The model under review builds one solid part; all positions refer to its coordinate system, in mm. A direction names the side the tool comes from. Give positions to 0.01 mm unless a question says otherwise; leave off trailing zeros. Loops run counter-clockwise (first coordinate to the right, second up) from the corner with the lowest first, then second, coordinate; pieces in that order, holes last. Notation, with made-up numbers: (-30, -17.75) -> (5, -17.75) arc R24 cw to (5, -2.75) -> close; hole circle Ø6 at (13, 6). An arc over 180 degrees is marked (long way). Write each question's results on one line, items separated by ' | '. Start each with the question number.
Q1. We need section C-C (y = 65.5). Write out the cut boundary in (x, z), plus the area to 3 significant figures.
Q2. Mouldability with a two-part tool opening along Z and no side actions: class faces 4 (the face through (2, 0, 67)), 5 (the face through (-59.37, 17.26, 143.18)), 6 (the face through (-105.034, 7.605, -66.17)) as released by +Z, released by -Z, zero draft, split by the parting line, or undercut.
Q3. We need section B-B (z = -112.5). Write out the cut boundary in (x, y).
Q4. Wall thickness on L1, parallel to X at y = 23, z = -1; L2, parallel to X at y = 77, z = 0; L3, parallel to X at y = 11.5, z = 0: over which ranges is each line inside the solid? List them lowest first. Write a range as [from, to].
Q5. We need section D-D (z = -56.25). Write out the cut boundary in (x, y), plus the area to 3 significant figures.
Q6. Insertion check: pin 1 Ø2 at (x, z) = (-23.5, 120) entering from +Y; pin 2 Ø3 at (y, z) = (60.5, -43) entering from -X; pin 3 Ø8 at (x, y) = (-1.5, 49.5) entering from +Z. Each pin has a flat end and moves straight along its axis. Give the tip position at first contact, or say it passes through.
Q7. We need section A-A (x = 0). Give the number of separate pieces and of enclosed holes in the cut face, plus the area to 3 significant figures.
Q8. Machinability: for faces 1 (the face through (37, 98, 10)), 2 (the face through (2.64, 24.65, 59.94)), 3 (the face through (-65, 15, 65)), which of the approach directions +Z, -Z, +X, -X, +Y, -Y give a long, thin tool a straight path to every point of the face, cutting with its end or side? Answer none if there is none.
from build123d import *

# Parameters (mm, degrees)
FLANGE_RIM_SKETCH_R              = 155
FLANGE_RIM_SKETCH_R_2            = 150
FLANGE_RIM_310_DEPTH             = 35
FLANGE_BASE_SKETCH_R             = 150
FLANGE_BASE_DISC_DEPTH           = 15
MOUNTING_HOLES_SKETCH_R          = 12.5
MOUNTING_HOLES_6X_DEPTH          = 65
HUB_SHOULDER_SKETCH_R            = 80
HUB_SHOULDER_160_DEPTH           = 25
HUB_SKETCH_R                     = 75
HUB_150_DEPTH                    = 105
KEYED_BORE_WITH_KEYWAY_8X8_DEPTH = 142
RECESS_SKETCH_R                  = 60
RECESS_120_DEPTH                 = 50


with BuildPart() as part:
    # Flange Rim Sketch → Flange Rim Ø310 (new body)
    with BuildSketch(Plane(origin=(0, 0, 0), x_dir=(1, 0, 0), z_dir=(0, 1, 0))):
        with Locations(Location((0, 0, 0), (0, 0, 270))):
            Circle(FLANGE_RIM_SKETCH_R)
        with Locations(Location((0, 0, 0), (0, 0, 270))):
            Circle(FLANGE_RIM_SKETCH_R_2, mode=Mode.SUBTRACT)
    extrude(amount=FLANGE_RIM_310_DEPTH)

    # Flange Base Sketch → Flange Base Disc (add)
    with BuildSketch(Plane(origin=(0, 0, 0), x_dir=(1, 0, 0), z_dir=(0, 1, 0))):
        with Locations(Location((0, 0, 0), (0, 0, 270))):
            Circle(FLANGE_BASE_SKETCH_R)
    extrude(amount=FLANGE_BASE_DISC_DEPTH)

    # Mounting Holes Sketch → Mounting Holes 6x (cut)
    with BuildSketch(Plane(origin=(0, 15, 0), x_dir=(1, 0, 0), z_dir=(0, 1, 0))):
        with Locations(Location((0, 112.5, 0), (0, 0, 270))):
            Circle(MOUNTING_HOLES_SKETCH_R)
        with Locations(Location((97.427857926, 56.25, 0), (0, 0, 270))):
            Circle(MOUNTING_HOLES_SKETCH_R)
        with Locations(Location((97.427857926, -56.25, 0), (0, 0, 270))):
            Circle(MOUNTING_HOLES_SKETCH_R)
        with Locations(Location((0, -112.5, 0), (0, 0, 270))):
            Circle(MOUNTING_HOLES_SKETCH_R)
        with Locations(Location((-97.427857926, -56.25, 0), (0, 0, 270))):
            Circle(MOUNTING_HOLES_SKETCH_R)
        with Locations(Location((-97.427857926, 56.25, 0), (0, 0, 270))):
            Circle(MOUNTING_HOLES_SKETCH_R)
    extrude(amount=-MOUNTING_HOLES_6X_DEPTH, mode=Mode.SUBTRACT)

    # Hub Shoulder Sketch → Hub Shoulder Ø160 (add)
    with BuildSketch(Plane(origin=(0, 15, 0), x_dir=(1, 0, 0), z_dir=(0, 1, 0))):
        with Locations(Location((0, 0, 0), (0, 0, 270))):
            Circle(HUB_SHOULDER_SKETCH_R)
    extrude(amount=HUB_SHOULDER_160_DEPTH)

    # Hub Sketch → Hub Ø150 (add)
    with BuildSketch(Plane(origin=(0, 40, 0), x_dir=(1, 0, 0), z_dir=(0, 1, 0))):
        with Locations(Location((0, 0, 0), (0, 0, 270))):
            Circle(HUB_SKETCH_R)
    extrude(amount=HUB_150_DEPTH)

    # Keyed Bore Sketch → Keyed Bore with Keyway 8x8 (cut)
    with BuildSketch(Plane(origin=(0, 145, 0), x_dir=(1, 0, 0), z_dir=(0, 1, 0))):
        with BuildLine():
            Line((41.541019662, 10), (33.541019662, 10))
            ThreePointArc((33.541019662, 10), (-35, 0), (33.541019662, -10))
            Line((33.541019662, -10), (41.541019662, -10))
            Line((41.541019662, -10), (41.541019662, 10))
        make_face()
    extrude(amount=-KEYED_BORE_WITH_KEYWAY_8X8_DEPTH, mode=Mode.SUBTRACT)

    # Recess Sketch → Recess Ø120 (cut)
    with BuildSketch(Plane.XZ):
        with Locations(Location((0, 0, 0), (0, 0, 270))):
            Circle(RECESS_SKETCH_R)
    extrude(amount=-RECESS_120_DEPTH, mode=Mode.SUBTRACT)


solid = part.part
Output:
1) outline: circle Ø150 at (0, 0); hole (33.54, -10) -> (41.54, -10) -> (41.54, 10) -> (33.54, 10) arc R35 ccw (long way) to start | area: 13,700 mm2
2) face 4: zero draft | face 5: split by the parting line | face 6: undercut
3) outline: (-106.62, 0) -> (-12.5, 0) -> (-12.5, 15) -> (-99.22, 15) -> (-99.22, 35) -> (-106.62, 35) -> close; (12.5, 0) -> (106.62, 0) -> (106.62, 35) -> (99.22, 35) -> (99.22, 15) -> (12.5, 15) -> close
4) L1: [-155, -150], [-79.99, -59.99], [59.99, 79.99], [150, 155] | L2: [-75, -35], [41.54, 75] | L3: [-155, -60], [60, 155]
5) outline: (-144.43, 0) -> (-109.93, 0) -> (-109.93, 15) -> (-139.05, 15) -> (-139.05, 35) -> (-144.43, 35) -> close; (-84.93, 0) -> (-20.88, 0) -> (-20.88, 50) -> (20.88, 50) -> (20.88, 0) -> (84.93, 0) -> (84.93, 15) -> (56.89, 15) -> (56.89, 40) -> (49.61, 40) -> (49.61, 145) -> (-49.61, 145) -> (-49.61, 40) -> (-56.89, 40) -> (-56.89, 15) -> (-84.93, 15) -> close; (109.93, 0) -> (144.43, 0) -> (144.43, 35) -> (139.05, 35) -> (139.05, 15) -> (109.93, 15) -> close | area: 15,000 mm2
6) pin 1: y = 15 | pin 2: x = -62.47 | pin 3: z = 75
7) separate pieces: 4 | enclosed holes: 0 | area: 11,200 mm2
8) face 1: +Y, -Y | face 2: -Y | face 3: +Y
